Source: CAD feature listing. Evaluate the final solid. Frame: model axes, mm. Face numbers are marked on the shaded views. A direction names the side the tool comes from. Give positions to 0.01 mm unless a question says otherwise; leave off trailing zeros. Order: outer loops, then holes, each group sorted by start corner. A loop starts at its lowest first (then second) coordinate and runs counter-clockwise, first axis right, second up. Notation, with made-up numbers: (38, 59.5) - (74, 59.5) arc R8 cw to (74, 68.5) - close; hole circle Ø4 at (10.5, -28). An arc over 180 degrees is marked (long way). Use CSV: the item, a comma, the result in double quotes.
```python
from build123d import *

# Parameters (mm, degrees)
BASE_PLATE_SKETCH_W       = 50
BASE_PLATE_SKETCH_H       = 90
BASE_PLATE_90X50X10_DEPTH = 10
UPRIGHT_WEB_DEPTH         = 24
WEB_WINDOW_CUT_DEPTH      = 112.018016556
WEB_WINDOW_CUT_DEPTH_BACK = 100
WEB_WINDOW_SKETCH_W       = 12
WEB_WINDOW_SKETCH_H       = 20
CYLINDER_BOSS_SKETCH_R    = 20
CYLINDER_BOSS_DEPTH       = 26
BOSS_START                = -10
BOSS_END_SLOT_20X10_DEPTH = 10
TOP_NOTCH_CUT_DEPTH       = 11


with BuildPart() as part:
    # Base Plate Sketch → Base Plate 90x50x10 (new body)
    with BuildSketch(Plane(origin=(0, 0, 0), x_dir=(1, 0, 0), z_dir=(0, 1, 0))):
        Rectangle(BASE_PLATE_SKETCH_W, BASE_PLATE_SKETCH_H)
    extrude(amount=BASE_PLATE_90X50X10_DEPTH)

    # Upright Web Sketch → Upright Web (add)
    with BuildSketch(Plane.ZY.offset(25)):
        Polygon((-25, 60), (25, 60), (45, 10), (-45, 10), align=None)
    extrude(amount=-UPRIGHT_WEB_DEPTH)

    # Web Window Sketch → Web Window Cut (cut, two sides: drawn at the far end of the back side and taken through both)
    with BuildSketch(Plane(origin=(0, 0, -45), x_dir=(-1, 0, 0), z_dir=(0, 0, -1)).offset(-WEB_WINDOW_CUT_DEPTH_BACK)):
        with Locations((13, 35)):
            Rectangle(WEB_WINDOW_SKETCH_W, WEB_WINDOW_SKETCH_H)
    extrude(amount=WEB_WINDOW_CUT_DEPTH + WEB_WINDOW_CUT_DEPTH_BACK, mode=Mode.SUBTRACT)

    # Cylinder Boss Sketch → Cylinder Boss (add)
    with BuildSketch(Plane(origin=(-1, 0, 0), x_dir=(0, 0, -1), z_dir=(1, 0, 0))):
        with Locations(Location((0, 45, 0), (0, 0, 131.409622109))):
            Circle(CYLINDER_BOSS_SKETCH_R)
    extrude(amount=CYLINDER_BOSS_DEPTH)

    # Boss End Slot Sketch → Boss End Slot 20x10 (cut)
    with BuildSketch(Plane(origin=(25, 0, 0), x_dir=(0, 0, -1), z_dir=(1, 0, 0)).offset(BOSS_START)):
        with BuildLine():
            Line((-10, 45), (10, 45))
            Line((10, 45), (10, 27.679491924))
            ThreePointArc((10, 27.679491924), (0, 25), (-10, 27.679491924))
            Line((-10, 27.679491924), (-10, 45))
        make_face()
    extrude(amount=BOSS_END_SLOT_20X10_DEPTH, mode=Mode.SUBTRACT)

    # Top Notch Sketch → Top Notch Cut (cut)
    with BuildSketch(Plane.ZY.offset(1)):
        with BuildLine():
            Line((-13.228756555, 60), (13.228756555, 60))
            ThreePointArc((13.228756555, 60), (0, 65), (-13.228756555, 60))
        make_face()
    extrude(amount=-TOP_NOTCH_CUT_DEPTH, mode=Mode.SUBTRACT)


solid = part.part
```
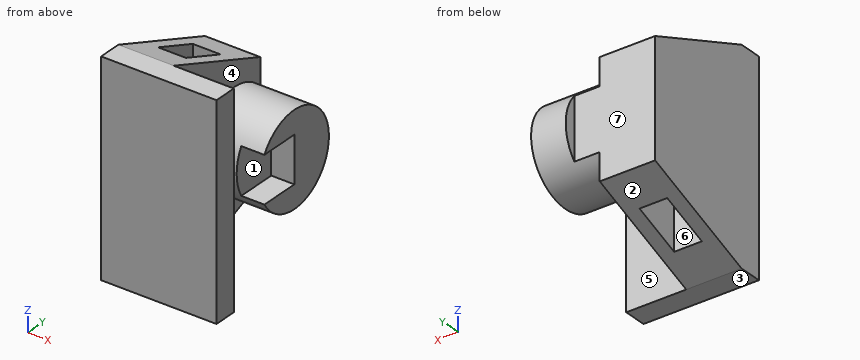
Item 1: Mould query, pull axis Y, two halves, no side actions, for the marked faces 1, 2 and 3. Classes: released by +Y, released by -Y, zero draft, split by the parting line, or undercut.
Filled in:
face 1,"undercut"
face 2,"released by +Y"
face 3,"zero draft"
Item 2: Material intervals for line 1 (X direction, y = 26, z = 25); line 2 (Y direction, x = -11, z = -17); line 3 (X direction, y = 34, z = 8), sorted ascending. Write a range as from..to.
Filled in:
line 1,"x = -25..-19, -7..-1"
line 2,"y = 0..25, 45..60"
line 3,"x = -25..-19, -7..15"
Item 3: Section D-D on z = 0. Return the cut outline in (x, y).
Filled in:
outline,"(-25, 0) - (25, 0) - (25, 10) - (-1, 10) - (-1, 25) - (15, 25) - (15, 45) - (25, 45) - (25, 65) - (10, 65) - (10, 60) - (-25, 60) - close; hole (-19, 25) - (-7, 25) - (-7, 45) - (-19, 45) - close"
Item 4: Set-up query: the marked faces 4, 5, 6 and 7. Return all of +Z, -Z, +X, -X, +Y, -Y with unobstructed straight access to the full face (end or side cutting, diameter ignored); none if empty.
Filled in:
face 4,"+X"
face 5,"+Z, -Z, +X"
face 6,"+Z, -Z"
face 7,"+Z, -Z, -X, +Y"
Item 5: Section B-B on z = -21.5. Return the cut outline in (x, y).
Filled in:
outline,"(-25, 0) - (25, 0) - (25, 10) - (-1, 10) - (-1, 60) - (-25, 60) - close; hole (-19, 25) - (-7, 25) - (-7, 45) - (-19, 45) - close"
Item 6: First-contact query: pin 1 (5 mm diameter, centred on x = 18.5, y = 36.5, fed in from +Z); pin 2 (16 mm diameter, centred on y = 33, z = 3, fed in from +X); pin 3 (1 mm diameter, centred on x = 10, y = 42.5, fed in from -Z); pin 4 (2 mm diameter, centred on x = -5.5, z = -10, fed in from +Y). Flat tips, straight axial feed; report the tip coordinate or a pass-through.
Filled in:
pin 1,"stops at z = 19.08"
pin 2,"stops at x = 25"
pin 3,"stops at z = -19.9"
pin 4,"stops at y = 60"
Item 7: Section A-A on y = 33. Return the cut outline in (x, z), then the cut area to 3 significant figures.
Filled in:
outline,"(-25, -35.8) - (-19, -35.8) - (-19, 35.8) - (-25, 35.8) - close; (-7, -35.8) - (-1, -35.8) - (-1, -16) - (25, -16) - (25, -10) - (15, -10) - (15, 10) - (25, 10) - (25, 16) - (-1, 16) - (-1, 35.8) - (-7, 35.8) - close"
area,"1,490 mm2"
Item 8: Section C-C on x = -11. Return the cut outline in (y, z).
Filled in:
outline,"(0, -45) - (10, -45) - (25, -39) - (25, 39) - (10, 45) - (0, 45) - close; (45, -31) - (60, -25) - (60, 25) - (45, 31) - close"
